The listing builds one solid part. Answer for the finished solid, in the listing's coordinates (mm). Face numbers are marked on the shaded views. Give positions to 0.01 mm unless a question says otherwise; leave off trailing zeros. Loops run counter-clockwise (first coordinate to the right, second up) from the corner with the lowest first, then second, coordinate; pieces in that order, holes last. Notation, with made-up numbers: M -1.5,-2 L 26.5,-2 A14 ccw 26.5,8 Z; hole C 14,-33 d10. An arc over 180 degrees is marked long. Return JSON: item names as keys, results as strings.
from build123d import *

# Parameters (mm, degrees)
SKETCH_1_W          = 75
SKETCH_1_H          = 55
EXTRUDE_1_DEPTH     = 50
SKETCH_2_W          = 65
SKETCH_2_H          = 45
CUT_EXTRUDE_1_DEPTH = 3
FILLET_1_R          = 3
FILLET_2_R          = 1


with BuildPart() as part:
    # 草图1 → 凸台-拉伸1 (new body)
    with BuildSketch(Plane.XY):
        with Locations((37.5, 27.5)):
            Rectangle(SKETCH_1_W, SKETCH_1_H)
    extrude(amount=EXTRUDE_1_DEPTH)

    # 草图2 → 切除-拉伸1 (cut)
    with BuildSketch(Plane.XY.offset(50)):
        with Locations((37.5, 27.5)):
            Rectangle(SKETCH_2_W, SKETCH_2_H)
    extrude(amount=-CUT_EXTRUDE_1_DEPTH, mode=Mode.SUBTRACT)

    # 圆角1
    fillet_1_edges = [part.edges().sort_by_distance(p)[0] for p in [
        (5, 5, 48.5),
        (5, 50, 48.5),
        (70, 50, 48.5),
        (70, 5, 48.5),
    ]]
    fillet(fillet_1_edges, radius=FILLET_1_R)

    # 圆角2
    fillet_2_edges = [part.edges().sort_by_distance(p)[0] for p in [
        (75, 27.5, 50),
        (37.5, 55, 50),
        (0, 27.5, 50),
        (37.5, 55, 0),
        (75, 27.5, 0),
        (37.5, 0, 0),
        (0, 27.5, 0),
        (0, 55, 25),
        (75, 55, 25),
        (75, 0, 25),
        (0, 0, 25),
        (37.5, 0, 50),
    ]]
    fillet(fillet_2_edges, radius=FILLET_2_R)


solid = part.part
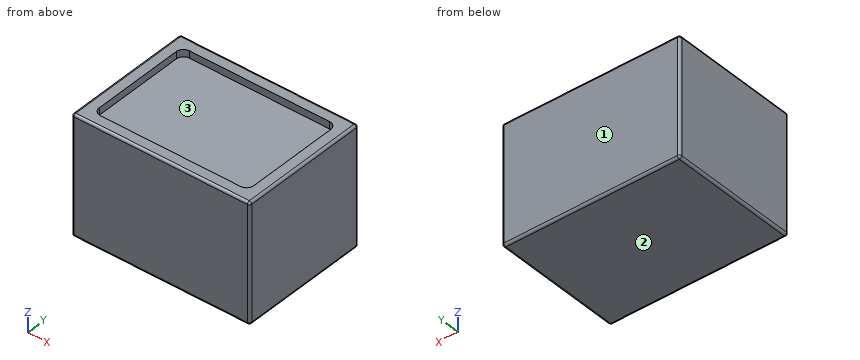
(1) Given pin 1 (2 mm diameter, centred on x = 49.5, y = 25.5, fed in from +Z), flat-ended and moving along its own axis, determine where the tip first touches the part or whether it passes through.
Values follow:
{"pin 1": "z = 47"}
(2) The part is cut by section A-A (y = 35.5). Determine the outline of the cut face in (x, z).
Values follow:
{"outline": "M 0,1 A1 ccw 1,0 L 74,0 A1 ccw 75,1 L 75,49 A1 ccw 74,50 L 70,50 L 70,47 L 5,47 L 5,50 L 1,50 A1 ccw 0,49 Z"}
(3) A straight line is drawn through the part: line 1 along Z through (x, y) = (30, 21). Find the intervals that lie inside material, in ascending order.
Values follow:
{"line 1": "0 to 47"}
(4) Determine the mould class of the marked faces 1, 2 and 3 for opening direction Y: released by +Y, released by -Y, zero draft, split by the parting line, or undercut.
Values follow:
{"face 1": "released by +Y", "face 2": "zero draft", "face 3": "undercut"}
(5) The part is cut by section B-B (x = 33). Determine the outline of the cut face in (y, z), and give its area (3 significant figures).
Values follow:
{"outline": "M 0,1 A1 ccw 1,0 L 54,0 A1 ccw 55,1 L 55,49 A1 ccw 54,50 L 50,50 L 50,47 L 5,47 L 5,50 L 1,50 A1 ccw 0,49 Z", "area": "2,610 mm²"}
